Here's how the part is built. I have some questions about the finished solid (model axes, mm). Round coordinates to 2 decimals unless told otherwise and drop trailing zeros. Write each loop counter-clockwise with the first axis right and the second up, starting at its lowest first coordinate (ties: lowest second). Pieces come first, ordered by that corner, then holes. Notation, with made-up numbers: (57, 89) -> (78, 89) arc R37 cw to (78, 126) -> close; hole circle Ø3 at (17.25, 56). An arc over 180 degrees is marked (long way). Answer in a Markdown table with one row per item. Add a question column.
from build123d import *

# Parameters (mm, degrees)
BOSS_EXTRUDE1_DEPTH = 475
FILLET1_R           = 100


with BuildPart() as part:
    # Sketch1 → Boss-Extrude1 (new body)
    with BuildSketch(Plane(origin=(0, 0, 0), x_dir=(1, 0, 0), z_dir=(0, 1, 0))):
        Polygon((0, 0), (279.136209435, 286.501268029), (662.731460294, 399.879764751), (659.896997876, 409.469646022), (273.796619493, 295.350713666), (-7.162531701, 6.978405236), align=None)
    extrude(amount=BOSS_EXTRUDE1_DEPTH)

    # Fillet1
    fillet1_edges = [part.edges().sort_by_distance(p)[0] for p in [
        (273.796619493, 237.5, -295.350713666),
        (279.136209435, 237.5, -286.501268029),
    ]]
    fillet(fillet1_edges, radius=FILLET1_R)


solid = part.part
Item 1: I need wall thicknesses on line 1 along Z through (x, y) = (571.5, 31.5); line 2 along Z through (x, y) = (527, 368); line 3 along X through (y, z) = (251.5, -76.5). Which ranges of each line are inside material? Lowest first, please. Write a range as from..to.
Item 2: If we section it at B-B on x = 187: Please give me the cut outline in (y, z), then the cut area to 3 significant figures.
Item 3: If we section it at C-C on z = -323: Please give me the cut outline in (x, y), then the cut area to 3 significant figures.
Item 4: For P1, Ø1.5, axis at x = 373, y = 372.5, coming from the -Z side; P2, Ø6, axis at x = 110, y = 403, coming from the -Z side; P3, Ø1.5, axis at y = 328.5, z = -246, coming from the +X side, each with a flat end and sliding along its axis, tell me the tip position at first contact or that it passes through.
Item 5: If we section it at A-A on y = 253.5: Please give me the cut outline in (x, z), then the cut area to 3 significant figures.
Results list:
| question | item | result |
|---|---|---|
| 1 | line 1 | -383.34..-372.91 |
| 1 | line 2 | -370.19..-359.76 |
| 1 | line 3 | 60.57..74.53 |
| 2 | outline | (0, -206.26) -> (475, -206.26) -> (475, -191.93) -> (0, -191.93) -> close |
| 2 | area | 6,810 mm² |
| 3 | outline | (367.34, 0) -> (402.62, 0) -> (402.62, 475) -> (367.34, 475) -> close |
| 3 | area | 16,800 mm² |
| 4 | P1 | z = -324.89 |
| 4 | P2 | z = -130.31 |
| 4 | P3 | x = 240.41 |
| 5 | outline | (-7.16, -6.98) -> (255.57, -276.64) arc R100 ccw to (298.85, -302.76) -> (659.9, -409.47) -> (662.73, -399.88) -> (304.19, -293.91) arc R100 cw to (260.91, -267.79) -> (0, 0) -> close |
| 5 | area | 8,030 mm² |
